```python
from build123d import *

# Parameters (mm, degrees)
SKETCH1_W               = 100
SKETCH1_H               = 98.830024952
SKETCH1_R               = 4.5
SKETCH1_W_2             = 60
SKETCH1_H_2             = 63.830024952
BOSS_EXTRUDE1_DEPTH     = 8
SKETCH4_R               = 5.55
CUT_EXTRUDE2_DEPTH      = 5
FILLET2_R               = 8
M2_5_TAPPED_HOLE1_D     = 2.05
M2_5_TAPPED_HOLE1_DEPTH = 6
M2_5_TAPPED_HOLE1_TIP   = 0.615882135
SKETCH11_R              = 1
CUT_EXTRUDE3_DEPTH      = 10
M4_TAPPED_HOLE1_D       = 3.3
M4_TAPPED_HOLE1_DEPTH   = 11.5
M4_TAPPED_HOLE1_TIP     = 0.991420021
SKETCH21_W              = 8
SKETCH21_H              = 10
BOSS_EXTRUDE2_DEPTH     = 50
M4_TAPPED_HOLE5_D       = 3.3
M4_TAPPED_HOLE5_DEPTH   = 8
M4_TAPPED_HOLE5_TIP     = 0.991420021
M4_TAPPED_HOLE6_D       = 3.3
M4_TAPPED_HOLE6_DEPTH   = 8
M4_TAPPED_HOLE6_TIP     = 0.991420021


with BuildPart() as part:
    # Sketch1 → Boss-Extrude1 (new body)
    with BuildSketch(Plane(origin=(0, 0, 0), x_dir=(0, 0, -1), z_dir=(1, 0, 0))):
        with Locations((9.943041263, -14.350886945)):
            Rectangle(SKETCH1_W, SKETCH1_H)
        with Locations((-30.056958737, 1.234100579)):
            Circle(SKETCH1_R, mode=Mode.SUBTRACT)
        with Locations((18.400547501, 25.064125531)):
            Circle(SKETCH1_R, mode=Mode.SUBTRACT)
        with Locations((49.943041263, -18.765899421)):
            Circle(SKETCH1_R, mode=Mode.SUBTRACT)
        with Locations((9.943041263, -16.850886945)):
            Rectangle(SKETCH1_W_2, SKETCH1_H_2, mode=Mode.SUBTRACT)
    extrude(amount=BOSS_EXTRUDE1_DEPTH)

    # Sketch4 → Cut-Extrude2 (cut)
    with BuildSketch(Plane.ZY):
        with Locations((-18.400547501, 25.064125531)):
            Circle(SKETCH4_R)
        with Locations((30.056958737, 1.234100579)):
            Circle(SKETCH4_R)
        with Locations((-49.943041263, -18.765899421)):
            Circle(SKETCH4_R)
    extrude(amount=-CUT_EXTRUDE2_DEPTH, mode=Mode.SUBTRACT)

    # Fillet2
    fillet2_edges = [part.edges().sort_by_distance(p)[0] for p in [
        (4, 15.064125531, 20.056958737),
        (4, -48.765899421, 20.056958737),
        (4, -48.765899421, -39.943041263),
        (4, 15.064125531, -39.943041263),
    ]]
    fillet(fillet2_edges, radius=FILLET2_R)

    # M2.5 Tapped Hole1
    with Locations(Plane(origin=(0, 25.064125531, -26.150547501), x_dir=(0, 0, -1), z_dir=(-1, 0, 0))):
        with Locations((0, 0), (-15.5, 0), (23.792493762, 36.080024952), (23.792493762, 51.580024952), (-56.207506238, 16.080024952), (-56.207506238, 31.580024952)):
            Hole(M2_5_TAPPED_HOLE1_D / 2, depth=M2_5_TAPPED_HOLE1_DEPTH)
            with Locations((0, 0, -(M2_5_TAPPED_HOLE1_DEPTH + M2_5_TAPPED_HOLE1_TIP / 2))):  # 118° drill point
                Cone(0, M2_5_TAPPED_HOLE1_D / 2, M2_5_TAPPED_HOLE1_TIP, mode=Mode.SUBTRACT)

    # Sketch11 → Cut-Extrude3 (cut)
    with BuildSketch(Plane.XZ.offset(63.765899421)):
        with Locations(Location((4.001919783, -44.943041263, 0), (0, 0, 270))):
            Circle(SKETCH11_R)
        with Locations(Location((4.001919783, 30.056958737, 0), (0, 0, 270))):
            Circle(SKETCH11_R)
        with Locations(Location((4.001919783, -19.943041263, 0), (0, 0, 270))):
            Circle(SKETCH11_R)
        with Locations(Location((4.001919783, 5.056958737, 0), (0, 0, 270))):
            Circle(SKETCH11_R)
    extrude(amount=-CUT_EXTRUDE3_DEPTH, mode=Mode.SUBTRACT)

    # M4 Tapped Hole1
    with Locations(Plane(origin=(0, -63.765899421, 0), x_dir=(-1, 0, 0), z_dir=(0, -1, 0))):
        with Locations((-4.001919783, 44.943041263), (-4.001919783, 19.943041263), (-4.001919783, -5.056958737), (-4.001919783, -30.056958737)):
            Hole(M4_TAPPED_HOLE1_D / 2, depth=M4_TAPPED_HOLE1_DEPTH)
            with Locations((0, 0, -(M4_TAPPED_HOLE1_DEPTH + M4_TAPPED_HOLE1_TIP / 2))):  # 118° drill point
                Cone(0, M4_TAPPED_HOLE1_D / 2, M4_TAPPED_HOLE1_TIP, mode=Mode.SUBTRACT)

    # Sketch21 → Boss-Extrude2 (add)
    with BuildSketch(Plane(origin=(0, 35.064125531, 0), x_dir=(1, 0, 0), z_dir=(0, 1, 0))):
        with Locations((4, 54.943041263)):
            Rectangle(SKETCH21_W, SKETCH21_H)
        with Locations((4, -35.056958737)):
            Rectangle(SKETCH21_W, SKETCH21_H)
    extrude(amount=BOSS_EXTRUDE2_DEPTH)

    # M4 Tapped Hole5
    with Locations(Plane(origin=(0, 85.064125531, 0), x_dir=(1, 0, 0), z_dir=(0, 1, 0))):
        with Locations((4, 54.943041263), (4, -35.056958737)):
            Hole(M4_TAPPED_HOLE5_D / 2, depth=M4_TAPPED_HOLE5_DEPTH)
            with Locations((0, 0, -(M4_TAPPED_HOLE5_DEPTH + M4_TAPPED_HOLE5_TIP / 2))):  # 118° drill point
                Cone(0, M4_TAPPED_HOLE5_D / 2, M4_TAPPED_HOLE5_TIP, mode=Mode.SUBTRACT)

    # M4 Tapped Hole6
    with Locations(Plane(origin=(0, 35.064125531, 0), x_dir=(1, 0, 0), z_dir=(0, 1, 0))):
        with Locations((4, 34.943041263), (4, -15.056958737)):
            Hole(M4_TAPPED_HOLE6_D / 2, depth=M4_TAPPED_HOLE6_DEPTH)
            with Locations((0, 0, -(M4_TAPPED_HOLE6_DEPTH + M4_TAPPED_HOLE6_TIP / 2))):  # 118° drill point
                Cone(0, M4_TAPPED_HOLE6_D / 2, M4_TAPPED_HOLE6_TIP, mode=Mode.SUBTRACT)


solid = part.part
```
Model file for the job. Use its own axes, mm. A direction names the side the tool comes from. Give positions to 0.01 mm unless a question says otherwise; leave off trailing zeros. Order: outer loops, then holes, each group sorted by start corner. A loop starts at its lowest first (then second) coordinate and runs counter-clockwise, first axis right, second up.
1) Wall check: probe 1 along Z at (x, y) = (4, 79); probe 2 along Z at (x, y) = (5, 41.5); probe 3 along Z at (x, y) = (4, 29). Give the ranges that are in metal, low to high.
2) Saw through at A-A, the plane z = -30.5. Write the cut outline in (x, y), then the cut area to 3 significant figures.
3) Saw through at B-B, the plane y = 73. Write the cut outline in (x, z).
4) Mould opens along Y. For faces 6 (the cylindrical face through (4.358, 81.008, 36.668)), 7 (the cylindrical face through (4.06, -46.48, -37.54)), 8 (the conical face through (3.938, 76.245, 35.337)), 9 (the flat face through (4, -63.766, -9)) say: +Y half, -Y half, draft (parallel to the pull), parting line (faces both ways), or undercut.
5) Pin check, flat tips, straight feed: pin 1 (4 mm diameter, centred on x = 4, z = 15.06, fed in from +Y); pin 2 (2.5 mm diameter, centred on x = 4, z = -44.94, fed in from -Y). Stop position of each tip, or through.
6) 3-axis set-ups, long thin cutter, end or side, ignore diameter. For faces 1 (the cylindrical face through (2.465, -20.892, -44.816)), 2 (the cylindrical face through (2.79, -57.94, -21.06)), 3 (the flat face through (4, -17, 20.057)), 4 (the cylindrical face through (4.358, 81.008, -53.332)), 5 (the flat face through (4, 35.064, -9)): which of +Z, -Z, +X, -X, +Y, -Y reach the whole face in a straight line?
Computed:
1. probe 1: z = -59.94 to -56.59, -53.29 to -49.94, 30.06 to 33.41, 36.71 to 40.06
1. probe 2: z = -59.94 to -49.94, 30.06 to 40.06
1. probe 3: z = -59.94 to -36.59, -33.29 to -22.31, -14.49 to 13.41, 16.71 to 40.06
2. outline: (0, -63.77) - (8, -63.77) - (8, -48.77) - (0, -48.77) - close; (0, 15.06) - (8, 15.06) - (8, 35.06) - (0, 35.06) - close
2. area: 280 mm2
3. outline: (0, -59.94) - (8, -59.94) - (8, -49.94) - (0, -49.94) - close; (0, 30.06) - (8, 30.06) - (8, 40.06) - (0, 40.06) - close
4. face 6: draft
4. face 7: undercut
4. face 8: +Y half
4. face 9: -Y half
5. pin 1: stops at y = 35.06
5. pin 2: stops at y = -52.03
6. face 1: -X
6. face 2: -Y
6. face 3: +X, -X
6. face 4: +Y
6. face 5: +X, -X, +Y
